The figure shows three views and two pictorial views of one solid part (mm, origin at its lowest corner). Answer the questions. Give positions to 0.01 mm unless a question says otherwise; leave off trailing zeros. Loops run counter-clockwise (first coordinate to the right, second up) from the corner with the lowest first, then second, coordinate; pieces in that order, holes last. Notation, with made-up numbers: (54, 72.25) - (96, 72.25) arc R15 cw to (96, 87.25) - close; hole circle Ø1 at (-39.5, 81.25). An arc over 180 degrees is marked (long way). Use CSV: the item, a comma, the result in double quotes.
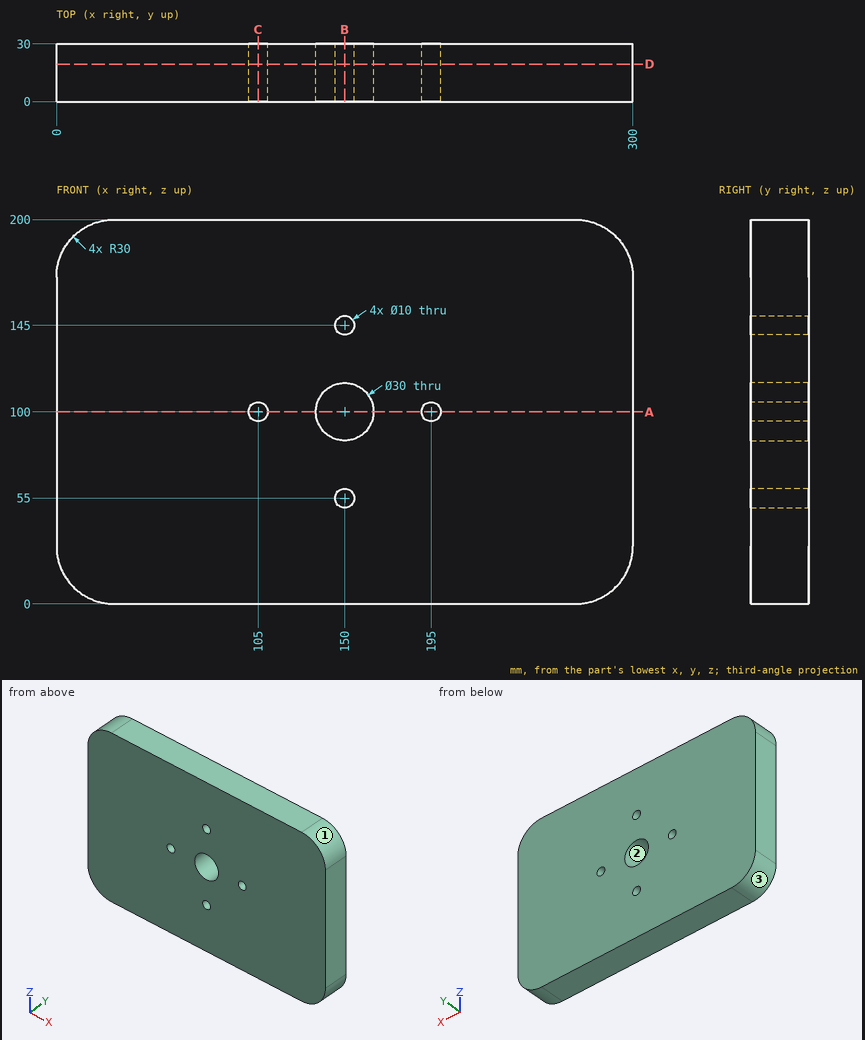
Item 1: A cutting plane is placed at C-C on x = 105. Determine the outline of the cut face in (y, z), and give its area (3 significant figures).
Determined:
outline,"(0, 0) - (30, 0) - (30, 95) - (0, 95) - close; (0, 105) - (30, 105) - (30, 200) - (0, 200) - close"
area,"5,700 mm²"
Item 2: Given P1, Ø3, axis at x = 72.5, z = 59.5, coming from the -Y side, flat-ended and moving along its own axis, determine where the tip first touches the part or whether it passes through.
Determined:
P1,"stops at y = 0"
Item 3: A cutting plane is placed at A-A on z = 100. Determine the outline of the cut face in (x, y), and give its area (3 significant figures).
Determined:
outline,"(0, 0) - (100, 0) - (100, 30) - (0, 30) - close; (110, 0) - (135, 0) - (135, 30) - (110, 30) - close; (165, 0) - (190, 0) - (190, 30) - (165, 30) - close; (200, 0) - (300, 0) - (300, 30) - (200, 30) - close"
area,"7,500 mm²"
Item 4: A cutting plane is placed at B-B on x = 150. Determine the outline of the cut face in (y, z), and give its area (3 significant figures).
Determined:
outline,"(0, 0) - (30, 0) - (30, 50) - (0, 50) - close; (0, 60) - (30, 60) - (30, 85) - (0, 85) - close; (0, 115) - (30, 115) - (30, 140) - (0, 140) - close; (0, 150) - (30, 150) - (30, 200) - (0, 200) - close"
area,"4,500 mm²"
Item 5: Find the intervals of material crossed by line 1 (X direction, y = 17.75, z = 100); line 2 (X direction, y = 24.25, z = 55); line 3 (Z direction, x = 141.5, y = 23.5), in increasing order.
Determined:
line 1,"x = 0 to 100, 110 to 135, 165 to 190, 200 to 300"
line 2,"x = 0 to 145, 155 to 300"
line 3,"z = 0 to 87.64, 112.36 to 200"
Item 6: A cutting plane is placed at D-D on y = 19.5. Determine the outline of the cut face in (x, z).
Determined:
outline,"(0, 30) arc R30 ccw to (30, 0) - (270, 0) arc R30 ccw to (300, 30) - (300, 170) arc R30 ccw to (270, 200) - (30, 200) arc R30 ccw to (0, 170) - close; hole circle Ø10 at (105, 100); hole circle Ø30 at (150, 100); hole circle Ø10 at (150, 55); hole circle Ø10 at (150, 145); hole circle Ø10 at (195, 100)"
Item 7: The mould has two halves that part along X. Classify the marked faces 1, 2 and 3: pulls with the +X half, pulls with the -X half, needs draft (parallel to the pull), parting line crosses it, or undercut.
Determined:
face 1,"pulls with the +X half"
face 2,"undercut"
face 3,"pulls with the -X half"
